Could you check a few things on this model? Use its own coordinates, in mm. Face numbers are marked on the shaded views. A direction names the side the tool comes from. Give positions to 0.01 mm unless a question says otherwise; leave off trailing zeros. Loops run counter-clockwise (first coordinate to the right, second up) from the corner with the lowest first, then second, coordinate; pieces in that order, holes last. Notation, with made-up numbers: (60, 15.25) - (119, 15.25) arc R12 ccw to (119, 29.25) - close; hole circle Ø2 at (66, 71.5). An arc over 180 degrees is marked (long way). Write each question's results on one line, items separated by ' | '. Start each with the question number.
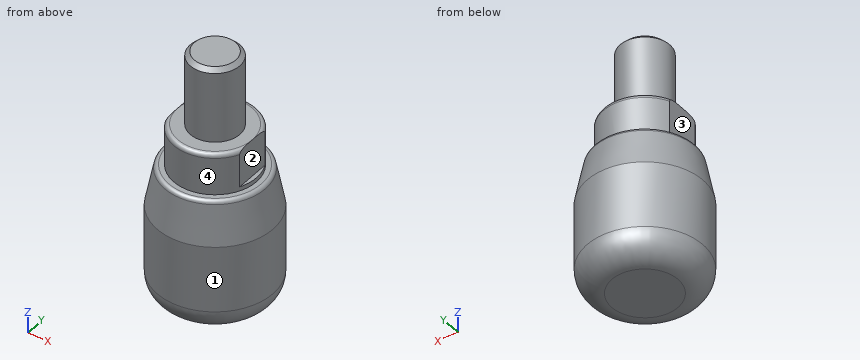
```python
from build123d import *

# Parameters (mm, degrees)
SKETCH1_R           = 7
BOSS_EXTRUDE1_DEPTH = 8
SKETCH2_R           = 5
BOSS_EXTRUDE2_DEPTH = 5
SKETCH3_R           = 3
BOSS_EXTRUDE3_DEPTH = 9
CHAMFER1_SIZE       = 5
CHAMFER1_SIZE2      = 1
FILLET1_R           = 3
FILLET2_R           = 0.5
FILLET3_R           = 0.5
SKETCH4_OUTSIDE_W   = 23.188
SKETCH4_OUTSIDE_H   = 23.188
SKETCH4_OUTSIDE_W_2 = 9
SKETCH4_OUTSIDE_H_2 = 10
CUT_EXTRUDE1_DEPTH  = 4.5
CHAMFER3_SIZE       = 0.5


with BuildPart() as part:
    # Sketch1 → Boss-Extrude1 (new, symmetric)
    with BuildSketch(Plane.XY):
        Circle(SKETCH1_R)
    extrude(amount=BOSS_EXTRUDE1_DEPTH, both=True)

    # Sketch2 → Boss-Extrude2 (add)
    with BuildSketch(Plane.XY.offset(8)):
        Circle(SKETCH2_R)
    extrude(amount=BOSS_EXTRUDE2_DEPTH)

    # Sketch3 → Boss-Extrude3 (add)
    with BuildSketch(Plane.XY.offset(13)):
        Circle(SKETCH3_R)
    extrude(amount=BOSS_EXTRUDE3_DEPTH)

    # Chamfer1
    chamfer1_edges = [part.edges().sort_by_distance(p)[0] for p in [
        (-7, 0, 8),
    ]]
    chamfer1_side = [part.faces().sort_by_distance(p)[0] for p in [
        (-7, 0, 0),
    ]]
    chamfer(chamfer1_edges, length=CHAMFER1_SIZE, length2=CHAMFER1_SIZE2, reference=chamfer1_side[0])

    # Fillet1
    fillet1_edges = [part.edges().sort_by_distance(p)[0] for p in [
        (-7, 0, -8),
    ]]
    fillet(fillet1_edges, radius=FILLET1_R)

    # Fillet2
    fillet2_edges = [part.edges().sort_by_distance(p)[0] for p in [
        (-6, 0, 8),
    ]]
    fillet(fillet2_edges, radius=FILLET2_R)

    # Fillet3
    fillet3_edges = [part.edges().sort_by_distance(p)[0] for p in [
        (-5, 0, 13),
    ]]
    fillet(fillet3_edges, radius=FILLET3_R)

    # Sketch4 outside → Cut-Extrude1 (cut)
    with BuildSketch(Plane.XY.offset(13)):
        Rectangle(SKETCH4_OUTSIDE_W, SKETCH4_OUTSIDE_H)
        Rectangle(SKETCH4_OUTSIDE_W_2, SKETCH4_OUTSIDE_H_2, mode=Mode.SUBTRACT)
    extrude(amount=-CUT_EXTRUDE1_DEPTH, mode=Mode.SUBTRACT)

    # Chamfer3
    chamfer3_edges = [part.edges().sort_by_distance(p)[0] for p in [
        (-3, 0, 22),
    ]]
    chamfer(chamfer3_edges, length=CHAMFER3_SIZE)


solid = part.part
```
Q1. I want a section at C-C, the plane z = 1.75. List the corners of the cut face in (x, y) for me, then the cut area to 3 significant figures.
Q2. I want a section at B-B, the plane z = 5.5. List the corners of the cut face in (x, y) for me, then the cut area to 3 significant figures.
Q3. I need wall thicknesses on L1, parallel to X at y = 2, z = 11.5; L2, parallel to Z at x = -4.75, y = 3; L3, parallel to Z at x = -3.75, y = -2.5. Which ranges of each line are inside material? Lowest first, please. Write a range as from..to.
Q4. Which directions (+Z, -Z, +X, -X, +Y, -Y) give clear straight access to the entire face, cutting with the end or side of a thin tool? Please do the marked faces 1, 2, 3 and 4.
Q5. I'm going to push flat-ended pins straight in: pin 1 Ø3 at (x, z) = (4.5, -4) entering from +Y; pin 2 Ø2 at (y, z) = (0.5, 11) entering from -X; pin 3 Ø5 at (x, y) = (5, 1.5) entering from +Z. Where does each tip first touch, or does it pass through?
Q6. I want a section at A-A, the plane x = 0. List the corners of the cut face in (y, z) for me, then the cut area to 3 significant figures.
Conclusion:
1) outline: circle Ø14 at (0, 0) | area: 154 mm^2
2) outline: circle Ø13 at (0, 0) | area: 133 mm^2
3) L1: -4.5..4.5 | L2: -7.53..8 | L3: -7.96..13
4) face 1: +Z, -Z | face 2: +Z, +X, +Y, -Y | face 3: +Z, -X, +Y, -Y | face 4: +Z
5) pin 1: y = 6.32 | pin 2: x = -4.5 | pin 3: z = 21.78
6) outline: (-7, -5) arc R3 ccw to (-4, -8) - (4, -8) arc R3 ccw to (7, -5) - (7, 3) - (6.08, 7.6) arc R0.5 ccw to (5.59, 8) - (5, 8) - (5, 12.5) arc R0.5 ccw to (4.5, 13) - (3, 13) - (3, 21.5) - (2.5, 22) - (-2.5, 22) - (-3, 21.5) - (-3, 13) - (-4.5, 13) arc R0.5 ccw to (-5, 12.5) - (-5, 8) - (-5.59, 8) arc R0.5 ccw to (-6.08, 7.6) - (-7, 3) - close | area: 319 mm^2
